Can you work these out from the drawing? Everything is in mm from the part's minimum corner. A direction names the side the tool comes from. Give positions to 0.01 mm unless a question says otherwise; leave off trailing zeros. Write each loop counter-clockwise with the first axis right and the second up, starting at its lowest first coordinate (ties: lowest second). Pieces come first, ordered by that corner, then holes. Notation, with made-up numbers: (11.5, 13) -> (68.5, 13) arc R28 ccw to (68.5, 35) -> close; hole circle Ø4 at (30.5, 30). An arc over 180 degrees is marked (long way). Write item = value, one per line. Start each with the question number.
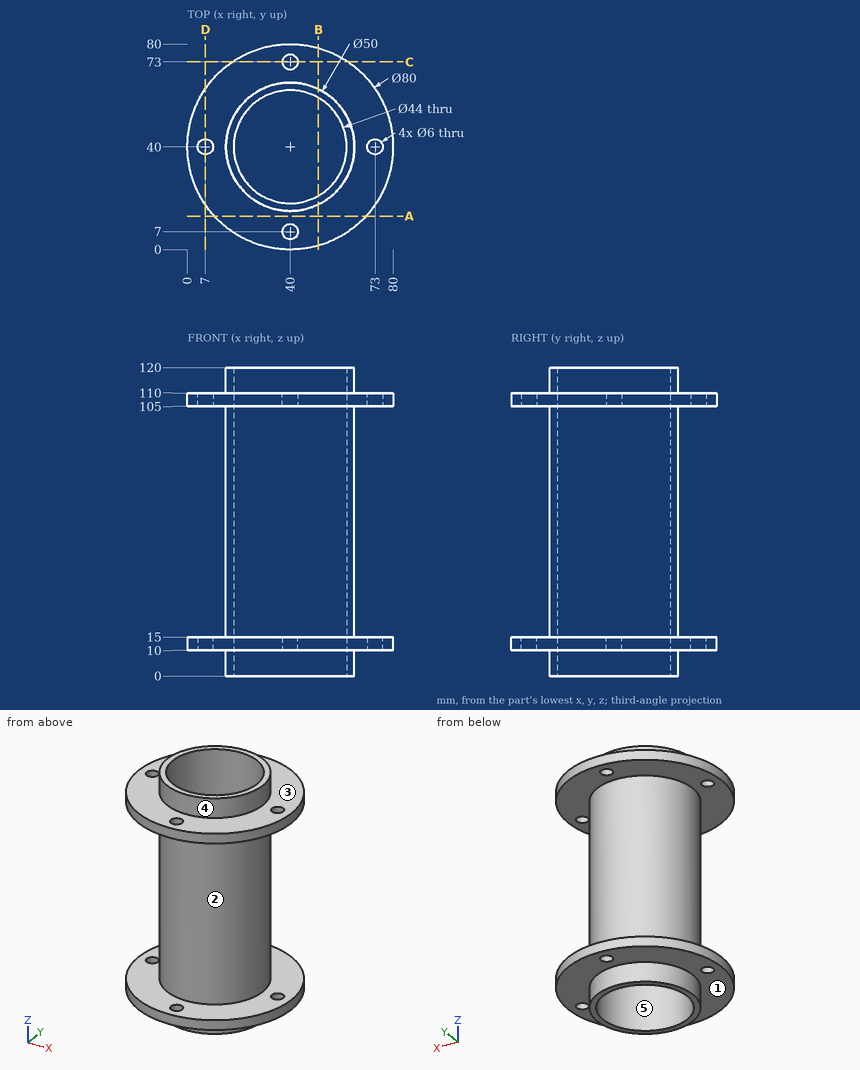
(1) Imagine slicing it at C-C (y = 73). Please give me the cut outline in (x, z), then the cut area to 3 significant figures.
(2) If I drill on line 1 along Y through (x, z) = (40, 13); line 2 along Z through (x, y) = (27.5, 62); line 3 along Y through (x, z) = (73, 106.9), over which ranges is the centre line in solid material (lowest first)? Write a range as from..to.
(3) I'm going to push flat-ended pins straight in: pin 1 (10 mm diameter, centred on x = 44, z = 19.5, fed in from +Y); pin 2 (10 mm diameter, centred on y = 69, z = 15.5, fed in from -X); pin 3 (2 mm diameter, centred on x = 63.5, z = 38.5, fed in from +Y); pin 4 (5.5 mm diameter, centred on x = 7, y = 40, fed in from +Z). Where does each tip first touch, or does it pass through?
(4) We'd pull the mould along X, two halves only. Please class the marked faces 3, 4 and 5: released by +X, released by -X, zero draft, split by the parting line, or undercut.
(5) On a 3-axis mill with a long thin cutter (end or side, diameter ignored), from which of +Z, -Z, +X, -X, +Y, -Y can I reach the whole of each face in a straight line? I mean the marked faces 1 and 2. Say none if no direction works.
(6) Imagine slicing it at A-A (y = 13). Please give me the cut outline in (x, z), then the cut area to 3 significant figures.
(7) Imagine slicing it at B-B (x = 51). Please give me the cut outline in (y, z).
Answers below:
q1.outline = (17.39, 10) -> (37, 10) -> (37, 15) -> (17.39, 15) -> close; (17.39, 105) -> (37, 105) -> (37, 110) -> (17.39, 110) -> close; (43, 10) -> (62.61, 10) -> (62.61, 15) -> (43, 15) -> close; (43, 105) -> (62.61, 105) -> (62.61, 110) -> (43, 110) -> close
q1.area = 392 mm^2
q2.line_1 = 0..4, 10..18, 62..70, 76..80
q2.line_2 = 10..15, 105..110
q2.line_3 = 17.39..37, 43..62.61
q3.pin_1 = 79.96
q3.pin_2 = 8.02
q3.pin_3 = 50.9
q3.pin_4 = through
q4.face_3 = zero draft
q4.face_4 = split by the parting line
q4.face_5 = undercut
q5.face_1 = -Z
q5.face_2 = none
q6.outline = (10.49, 10) -> (69.51, 10) -> (69.51, 15) -> (10.49, 15) -> close; (10.49, 105) -> (69.51, 105) -> (69.51, 110) -> (10.49, 110) -> close
q6.area = 590 mm^2
q7.outline = (1.54, 10) -> (17.55, 10) -> (17.55, 0) -> (20.95, 0) -> (20.95, 120) -> (17.55, 120) -> (17.55, 110) -> (1.54, 110) -> (1.54, 105) -> (17.55, 105) -> (17.55, 15) -> (1.54, 15) -> close; (59.05, 0) -> (62.45, 0) -> (62.45, 10) -> (78.46, 10) -> (78.46, 15) -> (62.45, 15) -> (62.45, 105) -> (78.46, 105) -> (78.46, 110) -> (62.45, 110) -> (62.45, 120) -> (59.05, 120) -> close
